Can you work these out from the model? Positions are in its coordinate system, mm. A direction names the side the tool comes from. Round coordinates to 2 decimals unless told otherwise and drop trailing zeros. Loops run counter-clockwise (first coordinate to the right, second up) from the corner with the lowest first, then second, coordinate; pieces in that order, holes last.
from build123d import *

# Parameters (mm, degrees)
G1_1_2_TAPPED_HOLE1_D     = 45.25
G1_1_2_TAPPED_HOLE1_DEPTH = 102.54
G1_1_2_TAPPED_HOLE1_TIP   = 13.594471505
CHAMFER1_SIZE             = 2


with BuildPart() as part:
    # Sketch1 → Revolve1 (revolve)
    with BuildSketch(Plane.XY, mode=Mode.PRIVATE) as revolve1_sk:
        Polygon((0, 0), (35, 0), (35, -12), (27.5, -12), (27.5, -20), (0, -20), align=None)
    revolve(revolve1_sk.sketch.rotate(Axis((0, -20, 0), (0, 1, 0)), 90), axis=Axis((0, -20, 0), (0, 1, 0)))

    # G1-1/2 Tapped Hole1
    with Locations(Plane(origin=(0, 0, 0), x_dir=(1, 0, 0), z_dir=(0, 1, 0))):
        with Locations((0, 0)):
            Hole(G1_1_2_TAPPED_HOLE1_D / 2, depth=G1_1_2_TAPPED_HOLE1_DEPTH)
            with Locations((0, 0, -(G1_1_2_TAPPED_HOLE1_DEPTH + G1_1_2_TAPPED_HOLE1_TIP / 2))):  # 118° drill point
                Cone(0, G1_1_2_TAPPED_HOLE1_D / 2, G1_1_2_TAPPED_HOLE1_TIP, mode=Mode.SUBTRACT)

    # Chamfer1
    chamfer1_edges = [part.edges().sort_by_distance(p)[0] for p in [
        (0, 0, 35),
    ]]
    chamfer(chamfer1_edges, length=CHAMFER1_SIZE)


solid = part.part
(1) If we section it at D-D, the plane y = -18.5: List the corners of the cut face in (x, z) for me (3 decimals).
Worked answers:
outline: circle Ø55 at (0, 0); hole circle Ø45.25 at (0, 0)
(2) If we section it at A-A, the plane x = 0: List the corners of the cut face in (y, z) for me (3 decimals), then the cut area to 3 significant figures.
Worked answers:
outline: (-20, -27.5) - (-12, -27.5) - (-12, -35) - (-2, -35) - (0, -33) - (0, -22.625) - (-20, -22.625) - close; (-20, 22.625) - (0, 22.625) - (0, 33) - (-2, 35) - (-12, 35) - (-12, 27.5) - (-20, 27.5) - close
area: 371 mm2
(3) Will these pins go through, and if not, where does the flat tip stop? P1, Ø2, axis at x = 22, y = -11.5, coming from the +Z side; P2, Ø5, axis at y = -11, z = -21.5, coming from the -X side; P3, Ø6, axis at y = -6, z = -9, coming from the +X side; P4, Ø3, axis at x = 14, z = -13.5, coming from the -Y side.
Worked answers:
P1: stops at z = 28
P2: stops at x = -29.39
P3: stops at x = 34.48
P4: passes through
(4) If we mould it in two halves opening along X, with no side actions, what happens to faces 1 (the flat face through (18, -12, 21)), 2 (the cylindrical face through (-21.58, -10.14, -6.8)), 3 (the conical face through (-9.95, -0.13, -31.6))? For each: released by +X, released by -X, zero draft, split by the parting line, or undercut.
Worked answers:
face 1: zero draft
face 2: undercut
face 3: split by the parting line
(5) If we section it at B-B, the plane z = 0: List the corners of the cut face in (x, y) for me (3 decimals), then the cut area to 3 significant figures.
Worked answers:
outline: (-35, -12) - (-27.5, -12) - (-27.5, -20) - (-22.625, -20) - (-22.625, 0) - (-33, 0) - (-35, -2) - close; (22.625, -20) - (27.5, -20) - (27.5, -12) - (35, -12) - (35, -2) - (33, 0) - (22.625, 0) - close
area: 371 mm2
(6) If I drill on line 1 (Y direction, x = 10.5, z = 28.5); line 2 (X direction, y = -15.75, z = 14.5); line 3 (X direction, y = -8.5, z = -5.5), over which ranges is the centre line in solid material (lowest first)?
Worked answers:
line 1: y = -12 to 0
line 2: x = -23.37 to -17.37, 17.37 to 23.37
line 3: x = -34.57 to -21.95, 21.95 to 34.57
(7) If we section it at C-C, the plane y = -6: List the corners of the cut face in (x, z) for me (3 decimals).
Worked answers:
outline: circle Ø70 at (0, 0); hole circle Ø45.25 at (0, 0)
(8) For faces 4 (the flat face through (22, 0, -8)), 5 (the cylindrical face through (24.397, -16.056, -12.69)), which set-ups out of +Z, -Z, +X, -X, +Y, -Y let a thin tool reach every point of the face, with its end or its side?
Worked answers:
face 4: +Z, -Z, +X, -X, +Y
face 5: -Y
